from build123d import *

# Parameters (mm, degrees)
SKETCH1_R           = 25
BOSS_EXTRUDE1_DEPTH = 160
SKETCH2_R           = 5
BOSS_EXTRUDE2_DEPTH = 20


with BuildPart() as part:
    # Sketch1 → Boss-Extrude1 (new body)
    with BuildSketch(Plane.XY):
        Circle(SKETCH1_R)
    extrude(amount=BOSS_EXTRUDE1_DEPTH)

    # Sketch2 → Boss-Extrude2 (add)
    with BuildSketch(Plane(origin=(0, 0, 0), x_dir=(-1, 0, 0), z_dir=(0, 0, -1))):
        Circle(SKETCH2_R)
    boss_extrude2 = extrude(amount=BOSS_EXTRUDE2_DEPTH)

    # Mirror1: Boss-Extrude2 across plane
    add(boss_extrude2.mirror(Plane(origin=(0, 0, 80), x_dir=(1, 0, 0), z_dir=(0, 0, -1))))


solid = part.part
Design review of the part built by this model. Coordinates are the model's own, in mm. A direction names the side the tool comes from. Round coordinates to 2 decimals unless told otherwise and drop trailing zeros. Write each loop counter-clockwise with the first axis right and the second up, starting at its lowest first coordinate (ties: lowest second). Pieces come first, ordered by that corner, then holes. Notation, with made-up numbers: (74, -27.5) - (114, -27.5) arc R25 ccw to (114, -13.5) - close; hole circle Ø8 at (-24, 36). An arc over 180 degrees is marked (long way). Use a Markdown table: item, result. Add a question column.
1. Wall thickness on probe 1 along Z at (x, y) = (-2.5, -22); probe 2 along Y at (x, z) = (1, 30); probe 3 along X at (y, z) = (-6.5, 91.5): over which ranges is each line inside the solid? List them lowest first.
2. Clearance check with flat-ended pins moving along their axes: pin 1 (1 mm diameter, centred on x = -1, y = -18, fed in from +Z); pin 2 (10 mm diameter, centred on y = 9.5, z = 29, fed in from -X); pin 3 (1 mm diameter, centred on x = -1.5, y = -9, fed in from -Z). State where each tip first meets the part, or that it passes through.
3. We need section A-A (y = 0). State the section outline as (x, z) points, then the cut area to 3 significant figures.
4. We need section C-C (z = 5). State the section outline as (x, y) points, then the cut area to 3 significant figures.
5. For faces 1 (the face through (23.846, 7.509, 78.88)), 2 (the face through (1.08, -4.88, 169.86)), 3 (the face through (1.08, -4.88, -9.86)), list the 3-axis set-ups (+Z, -Z, +X, -X, +Y, -Y) from which the entire face can be reached by the end or side of a thin tool; tool diameter is ignored.
6. We need section D-D (x = 20). State the section outline as (y, z) points.
Output:
| question | item | result |
|---|---|---|
| 1 | probe 1 | z = 0 to 160 |
| 1 | probe 2 | y = -24.98 to 24.98 |
| 1 | probe 3 | x = -24.14 to 24.14 |
| 2 | pin 1 | stops at z = 160 |
| 2 | pin 2 | stops at x = -24.59 |
| 2 | pin 3 | stops at z = 0 |
| 3 | outline | (-25, 0) - (-5, 0) - (-5, -20) - (5, -20) - (5, 0) - (25, 0) - (25, 160) - (5, 160) - (5, 180) - (-5, 180) - (-5, 160) - (-25, 160) - close |
| 3 | area | 8,400 mm2 |
| 4 | outline | circle Ø50 at (0, 0) |
| 4 | area | 1,960 mm2 |
| 5 | face 1 | +Z, -Z |
| 5 | face 2 | +Z |
| 5 | face 3 | -Z |
| 6 | outline | (-15, 0) - (15, 0) - (15, 160) - (-15, 160) - close |
